Geometry: final body of the model. Coordinates: model frame, mm. Face numbers are marked on the shaded views. A direction names the side the tool comes from. Give positions to 0.01 mm unless a question says otherwise; leave off trailing zeros. Write each loop counter-clockwise with the first axis right and the second up, starting at its lowest first coordinate (ties: lowest second). Pieces come first, ordered by that corner, then holes.
from build123d import *

# Parameters (mm, degrees)
SKETCH_2_R          = 12.35
CUT_EXTRUDE_1_DEPTH = 8


with BuildPart() as part:
    # 草图1 → 旋转1 (revolve)
    with BuildSketch(Plane.XY, mode=Mode.PRIVATE) as revolve_1_sk:
        with BuildLine():
            Line((128, 0), (128, -4.9265))
            Line((128, -4.9265), (126.9265, -6))
            Line((126.9265, -6), (28, -6))
            Line((28, -6), (28, -11.875))
            Line((28, -11.875), (21.461538462, -11.875))
            Line((21.461538462, -11.875), (20, -6))
            Line((20, -6), (20, -14))
            ThreePointArc((20, -14), (17.071067812, -21.071067812), (10, -24))
            Line((10, -24), (2, -24))
            Line((2, -24), (2, -30))
            Line((2, -30), (0, -30))
            Line((0, -30), (0, 0))
            Line((0, 0), (128, 0))
        make_face()
    revolve(revolve_1_sk.sketch.rotate(Axis((0, 0, 0), (1, 0, 0)), 180), axis=Axis((0, 0, 0), (1, 0, 0)))

    # 草图2 → 切除-拉伸1 (cut)
    with BuildSketch(Plane(origin=(28, 0, 0), x_dir=(0, 0, -1), z_dir=(1, 0, 0))):
        Circle(SKETCH_2_R)
        Polygon((-9.5, 5.484827557), (-9.5, -5.484827557), (0, -10.969655115), (9.5, -5.484827557), (9.5, 5.484827557), (0, 10.969655115), align=None, mode=Mode.SUBTRACT)
    extrude(amount=-CUT_EXTRUDE_1_DEPTH, mode=Mode.SUBTRACT)


solid = part.part
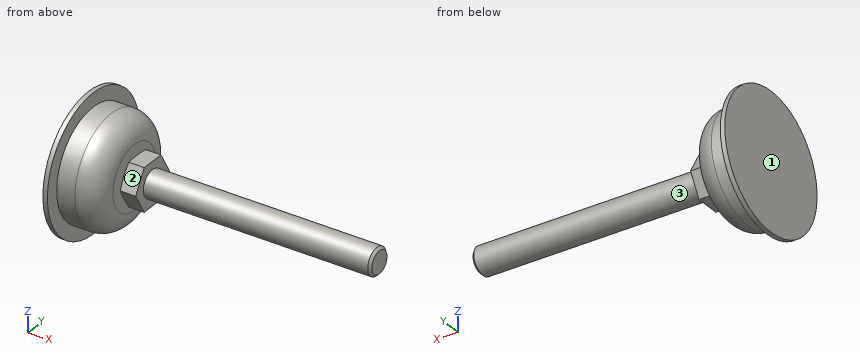
Q1. Access query for the marked faces 1, 2 and 3. Directions: +Z, -Z, +X, -X, +Y, -Y. A direction counts if a zero-diameter tool reaches every point of the face in a straight line with its end or side. Return the directions, or none.
Filled sheet:
face 1: +Z, -Z, -X, +Y, -Y
face 2: +Z, +X, -Y
face 3: +X
Q2. Ray query, line 1 along X through (y, z) = (25, -11); line 2 along Z through (x, y) = (22.5, 3.5); line 3 along X through (y, z) = (15, -9). Return the intervals inside material, ascending.
Filled sheet:
line 1: x = 0 to 2
line 2: z = -9.5 to 9.5
line 3: x = 0 to 19.37
Q3. Pin query (flat end, axial travel): P1, Ø2, axis at x = 25.5, y = 0.5, coming from the +Z side; P2, Ø2, axis at x = 25, y = -1, coming from the -Z side; P3, Ø10, axis at x = 68.5, z = 6, coming from the -Y side. Return the tip coordinate at first contact, or that it passes through.
Filled sheet:
P1: stops at z = 9.5
P2: stops at z = -9.5
P3: stops at y = -5.92
Q4. Section B-B on x = 23. Output: boundary loops of the cut face in (y, z), plus the area to 3 significant figures.
Filled sheet:
outline: (-10.97, 0) - (-5.48, -9.5) - (5.48, -9.5) - (10.97, 0) - (5.48, 9.5) - (-5.48, 9.5) - close
area: 313 mm2
Q5. Section A-A on y = 0. Output: boundary loops of the cut face in (x, z).
Filled sheet:
outline: (0, -30) - (2, -30) - (2, -24) - (10, -24) arc R10 ccw to (20, -14) - (20, -6) - (20.87, -9.5) - (28, -9.5) - (28, -6) - (126.93, -6) - (128, -4.93) - (128, 4.93) - (126.93, 6) - (28, 6) - (28, 9.5) - (20.87, 9.5) - (20, 6) - (20, 14) arc R10 ccw to (10, 24) - (2, 24) - (2, 30) - (0, 30) - close
